Design review of the part built by this model. Coordinates are the model's own, in mm. A direction names the side the tool comes from. Give positions to 0.01 mm unless a question says otherwise; leave off trailing zeros. Loops run counter-clockwise (first coordinate to the right, second up) from the corner with the lowest first, then second, coordinate; pieces in that order, holes last. Notation, with made-up numbers: (5, 75) - (56, 75) arc R38 ccw to (56, 113) - close; hole circle Ø10 at (30.5, 28). An arc over 180 degrees is marked (long way). Put each result on its own line as item: value. Start each with the question number.
```python
from build123d import *

# Parameters (mm, degrees)
SKETCH1_R                      = 7
BOSS_EXTRUDE1_DEPTH            = 30
SKETCH2_R                      = 25
BOSS_EXTRUDE2_DEPTH            = 3
SKETCH3_W                      = 60
SKETCH3_H                      = 60
BOSS_EXTRUDE3_DEPTH            = 6
BOSS_EXTRUDE4_DEPTH            = 115.5
SKETCH5_W                      = 35
SKETCH5_H                      = 25
BOSS_EXTRUDE5_DEPTH            = 12
CHAMFER1_SIZE                  = 10
CHAMFER1_SIZE2                 = 5.773502692
F_5_5_5_5_DIAMETER_HOLE1_D     = 5.5
F_5_5_5_5_DIAMETER_HOLE1_DEPTH = 20
F_5_5_5_5_DIAMETER_HOLE1_TIP   = 1.652366702
FILLET1_R                      = 5
SKETCH8_R                      = 5
BOSS_EXTRUDE6_DEPTH            = 6


with BuildPart() as part:
    # Sketch1 → Boss-Extrude1 (new body)
    with BuildSketch(Plane.XY):
        Circle(SKETCH1_R)
    extrude(amount=-BOSS_EXTRUDE1_DEPTH)

    # Sketch2 → Boss-Extrude2 (add)
    with BuildSketch(Plane(origin=(0, 0, -30), x_dir=(-1, 0, 0), z_dir=(0, 0, -1))):
        Circle(SKETCH2_R)
    extrude(amount=-BOSS_EXTRUDE2_DEPTH)

    # Sketch3 → Boss-Extrude3 (add)
    with BuildSketch(Plane(origin=(0, 0, -30), x_dir=(-1, 0, 0), z_dir=(0, 0, -1))):
        Rectangle(SKETCH3_W, SKETCH3_H)
    extrude(amount=BOSS_EXTRUDE3_DEPTH)

    # Sketch4 → Boss-Extrude4 (add)
    with BuildSketch(Plane(origin=(0, 0, -36), x_dir=(-1, 0, 0), z_dir=(0, 0, -1))):
        with BuildLine():
            Line((30, -17.5), (30, 17.5))
            ThreePointArc((30, 17.5), (21.161165235, 21.161165235), (17.5, 30))
            Line((17.5, 30), (-17.5, 30))
            ThreePointArc((-17.5, 30), (-21.161165235, 21.161165235), (-30, 17.5))
            Line((-30, 17.5), (-30, -17.5))
            ThreePointArc((-30, -17.5), (-21.161165235, -21.161165235), (-17.5, -30))
            Line((-17.5, -30), (17.5, -30))
            ThreePointArc((17.5, -30), (21.161165235, -21.161165235), (30, -17.5))
        make_face()
    extrude(amount=BOSS_EXTRUDE4_DEPTH)

    # Sketch5 → Boss-Extrude5 (add)
    with BuildSketch(Plane(origin=(0, 30, 0), x_dir=(1, 0, 0), z_dir=(0, 1, 0))):
        with Locations((0, 133)):
            Rectangle(SKETCH5_W, SKETCH5_H)
    extrude(amount=BOSS_EXTRUDE5_DEPTH)

    # Chamfer1
    chamfer1_edges = [part.edges().sort_by_distance(p)[0] for p in [
        (0, 42, -145.5),
    ]]
    chamfer1_side = [part.faces().sort_by_distance(p)[0] for p in [
        (0, 42, -133),
    ]]
    chamfer(chamfer1_edges, length=CHAMFER1_SIZE, length2=CHAMFER1_SIZE2, reference=chamfer1_side[0])

    # Ø5.5 (5.5) Diameter Hole1
    with Locations(Plane.XY.offset(-30)):
        with Locations((24.748737342, 24.748737342), (-24.748737342, 24.748737342), (24.748737342, -24.748737342), (-24.748737342, -24.748737342)):
            Hole(F_5_5_5_5_DIAMETER_HOLE1_D / 2, depth=F_5_5_5_5_DIAMETER_HOLE1_DEPTH)
            with Locations((0, 0, -(F_5_5_5_5_DIAMETER_HOLE1_DEPTH + F_5_5_5_5_DIAMETER_HOLE1_TIP / 2))):  # 118° drill point
                Cone(0, F_5_5_5_5_DIAMETER_HOLE1_D / 2, F_5_5_5_5_DIAMETER_HOLE1_TIP, mode=Mode.SUBTRACT)

    # Fillet1
    fillet1_edges = [part.edges().sort_by_distance(p)[0] for p in [
        (30, -30, -33),
        (-30, -30, -33),
        (-30, 30, -33),
        (30, 30, -33),
    ]]
    fillet(fillet1_edges, radius=FILLET1_R)

    # Sketch8 → Boss-Extrude6 (add)
    with BuildSketch(Plane(origin=(0, 0, -36), x_dir=(-1, 0, 0), z_dir=(0, 0, -1))):
        with Locations((-24.748737342, 24.748737342)):
            Circle(SKETCH8_R)
        with Locations((-24.748737342, -24.748737342)):
            Circle(SKETCH8_R)
        with Locations((24.748737342, -24.748737342)):
            Circle(SKETCH8_R)
        with Locations((24.748737342, 24.748737342)):
            Circle(SKETCH8_R)
    extrude(amount=BOSS_EXTRUDE6_DEPTH)


solid = part.part
```
Item 1: Consider section A-A (z = -115.5). State the section outline as (x, y) points, plus the area to 3 significant figures.
Item 2: Consider section B-B (x = 0). State the section outline as (y, z) points, plus the area to 3 significant figures.
Item 3: Consider section C-C (y = 13). State the section outline as (x, z) points.
Item 4: For P1, Ø3, axis at x = 22.5, y = -23, coming from the -Z side; P2, Ø4, axis at x = 8, z = -16.5, coming from the -Y side; P3, Ø1.8, axis at x = 1, z = -149, coming from the +Y side, all flat-tipped, find the tip position at first contact; note any pin that passes through.
Item 5: For L1, parallel to Y at x = -12, z = -39; L2, parallel to Z at x = 10, y = -15.5; L3, parallel to Z at x = 26.5, y = 7.5, list the stretches that pass through material, from the lowest coordinate up. Write a range as from..to.
Item 6: Mouldability with a two-part tool opening along X and no side actions: class faces 1 (the flat face through (0, 0, 0)), 2 (the flat face through (-17.5, 36, -133)), 3 (the cylindrical face through (-23.66, 19.87, -38.96)) as pulls with the +X half, pulls with the -X half, needs draft (parallel to the pull), parting line crosses it, or undercut.
Item 7: Machinability: for faces 4 (the flat face through (-19.6, -24.6, -36)), 5 (the flat face through (-25, 25, -42)), 6 (the flat face through (-25, -25, -36)), 7 (the flat face through (17.5, 36, -133)), which of the approach directions +Z, -Z, +X, -X, +Y, -Y give a long, thin tool a straight path to every point of the face, cutting with its end or side? Answer none if there is none.
Item 8: Consider section D-D (x = -12). State the section outline as (y, z) points.
Geometry says:
1. outline: (-30, -17.5) arc R12.5 cw to (-17.5, -30) - (17.5, -30) arc R12.5 cw to (30, -17.5) - (30, 17.5) arc R12.5 cw to (17.5, 30) - (-17.5, 30) arc R12.5 cw to (-30, 17.5) - close
1. area: 3,110 mm2
2. outline: (-30, -151.5) - (30, -151.5) - (30, -145.5) - (36.23, -145.5) - (42, -135.5) - (42, -120.5) - (30, -120.5) - (30, -30) - (25, -30) - (25, -27) - (7, -27) - (7, 0) - (-7, 0) - (-7, -27) - (-25, -27) - (-25, -30) - (-30, -30) - close
2. area: 8,090 mm2
3. outline: (-30, -151.5) - (30, -151.5) - (30, -30) - (21.35, -30) - (21.35, -27) - (-21.35, -27) - (-21.35, -30) - (-30, -30) - close
4. P1: stops at z = -42
4. P2: stops at y = -3.61
4. P3: stops at y = 30
5. L1: y = -30..30
5. L2: z = -151.5..-27
5. L3: z = -151.5..-30
6. face 1: needs draft
6. face 2: pulls with the -X half
6. face 3: undercut
7. face 4: -Z
7. face 5: -Z, -X, +Y
7. face 6: +Z
7. face 7: +Z, -Z, +X, +Y
8. outline: (-30, -151.5) - (30, -151.5) - (30, -145.5) - (36.23, -145.5) - (42, -135.5) - (42, -120.5) - (30, -120.5) - (30, -30) - (21.93, -30) - (21.93, -27) - (-21.93, -27) - (-21.93, -30) - (-30, -30) - close
